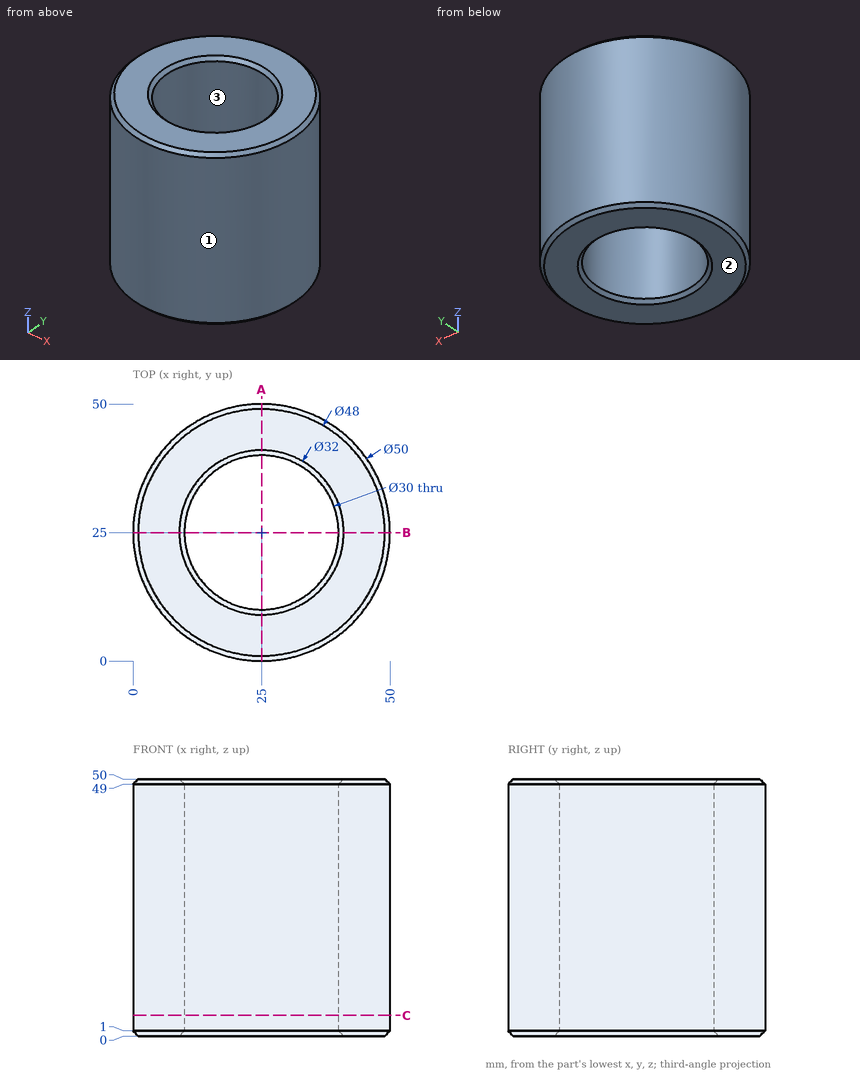
Part print with two shaded views. Sizes in mm from the minimum x, y, z corner. Round coordinates to 2 decimals unless told otherwise and drop trailing zeros. Write each loop counter-clockwise with the first axis right and the second up, starting at its lowest first coordinate (ties: lowest second). Pieces come first, ordered by that corner, then holes. Notation, with made-up numbers: M 10.25,61.5 L 30.25,61.5 A16 ccw 30.25,82.5 Z; hole C 74,-2 d1. An arc over 180 degrees is marked long. Put each result on its own line as item: value. Start each with the question number.
1) Saw through at C-C, the plane z = 4. Write the cut outline in (x, y).
2) Saw through at A-A, the plane x = 25. Write the cut outline in (y, z), and give its area (3 significant figures).
3) Pull direction Y, two halves, no side cores. Call the marked faces 1, 2 and 3: pulls with the +Y half, pulls with the -Y half, needs draft (parallel to the pull), parting line crosses it, or undercut.
4) Drill centre lines: probe 1 along Y at (x, z) = (25, 13.5); probe 2 along Y at (x, z) = (5, 45.5); probe 3 along Y at (x, z) = (34, 45). Where is each one in solid material? Low to high. Write a range as [from, to].
5) Pin check, flat tips, straight feed: pin 1 Ø1.5 at (x, z) = (18, 5.5) entering from -Y; pin 2 Ø1 at (x, y) = (14.5, 13) entering from -Z; pin 3 Ø8 at (x, z) = (14.5, 19) entering from -Y; pin 4 Ø2 at (x, z) = (14, 11.5) entering from +Y. Stop position of each tip, or through.
Resolved:
1. outline: C 25,25 d50; hole C 25,25 d30
2. outline: M 0,1 L 1,0 L 9,0 L 10,1 L 10,49 L 9,50 L 1,50 L 0,49 Z; M 40,1 L 41,0 L 49,0 L 50,1 L 50,49 L 49,50 L 41,50 L 40,49 Z
2. area: 996 mm²
3. face 1: parting line crosses it
3. face 2: needs draft
3. face 3: undercut
4. probe 1: [0, 10], [40, 50]
4. probe 2: [10, 40]
4. probe 3: [1.68, 13], [37, 48.32]
5. pin 1: y = 0.79
5. pin 2: z = 0
5. pin 3: y = 0.86
5. pin 4: y = 47.91
